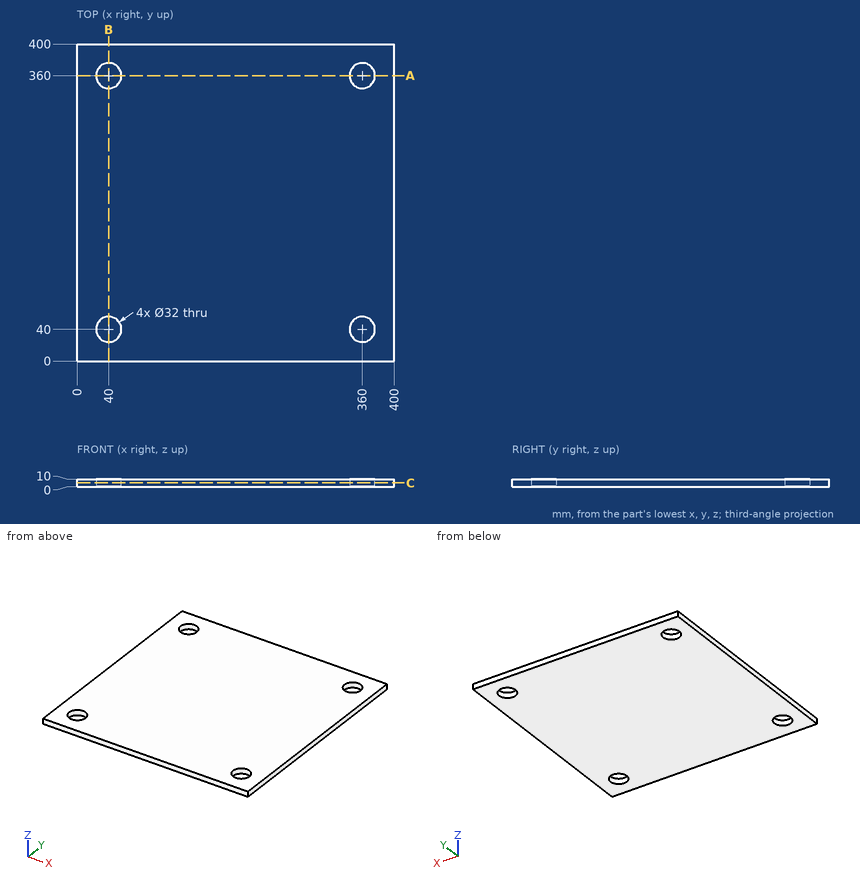
Geometry: see drawing. Coordinates: mm, zero at the bounding-box minimum. Give positions to 0.01 mm unless a question says otherwise; leave off trailing zeros. Loops run counter-clockwise (first coordinate to the right, second up) from the corner with the lowest first, then second, coordinate; pieces in that order, holes last. Notation, with made-up numbers: (64.25, 39.25) -> (103.25, 39.25) arc R27 cw to (103.25, 63.25) -> close; hole circle Ø2 at (79, 12.5). An arc over 180 degrees is marked (long way). Answer as a JSON object with one key per item and string values. Group by question number.
Item 1: Cut plane C-C, the plane z = 5.25. Return the cut outline in (x, y), and give its area (3 significant figures).
Item 2: Cut plane A-A, the plane y = 360. Return the cut outline in (x, z).
Item 3: Line query: probe 1 along Y at (x, z) = (40, 3.75); probe 2 along X at (y, z) = (29, 6.5). Output: solid intervals per line, ascending.
Checks:
{
 "1": {"outline": "(0, 0) -> (400, 0) -> (400, 400) -> (0, 400) -> close; hole circle Ø32 at (40, 40); hole circle Ø32 at (40, 360); hole circle Ø32 at (360, 40); hole circle Ø32 at (360, 360)", "area": "157,000 mm²"},
 "2": {"outline": "(0, 0) -> (24, 0) -> (24, 10) -> (0, 10) -> close; (56, 0) -> (344, 0) -> (344, 10) -> (56, 10) -> close; (376, 0) -> (400, 0) -> (400, 10) -> (376, 10) -> close"},
 "3": {"probe 1": "y = 0 to 24, 56 to 344, 376 to 400", "probe 2": "x = 0 to 28.38, 51.62 to 348.38, 371.62 to 400"}
}
